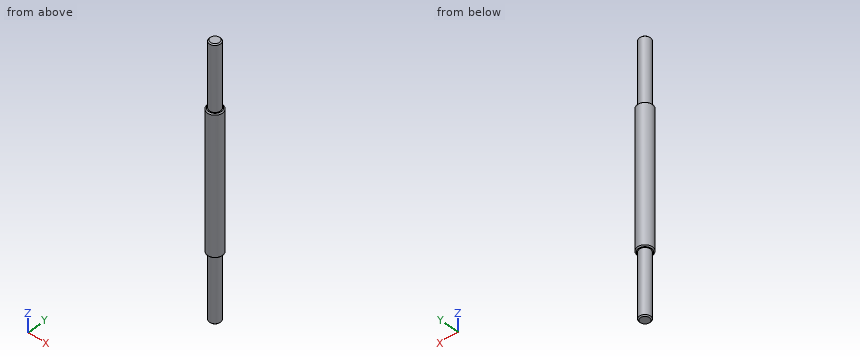
```python
from build123d import *

# Parameters (mm, degrees)
SKETCH1_R           = 7.5
BOSS_EXTRUDE1_DEPTH = 138
SKETCH2_R           = 5.5
BOSS_EXTRUDE2_DEPTH = 20
SKETCH3_R           = 5.5
BOSS_EXTRUDE3_DEPTH = 45
CHAMFER1_SIZE       = 1
BOSS_EXTRUDE4_START = 65
SKETCH4_R           = 5.5
BOSS_EXTRUDE4_DEPTH = 65
CHAMFER2_SIZE       = 1


with BuildPart() as part:
    # Sketch1 → Boss-Extrude1 (new body)
    with BuildSketch(Plane.XY):
        Circle(SKETCH1_R)
    extrude(amount=BOSS_EXTRUDE1_DEPTH)

    # Sketch2 → Boss-Extrude2 (add)
    with BuildSketch(Plane.XY.offset(138)):
        Circle(SKETCH2_R)
    extrude(amount=BOSS_EXTRUDE2_DEPTH)

    # Sketch3 → Boss-Extrude3 (add)
    with BuildSketch(Plane.XY.offset(158)):
        Circle(SKETCH3_R)
    extrude(amount=BOSS_EXTRUDE3_DEPTH)

    # Chamfer1
    chamfer1_edges = [part.edges().sort_by_distance(p)[0] for p in [
        (-7.5, 0, 0),
        (-7.5, 0, 138),
        (-5.5, 0, 203),
    ]]
    chamfer(chamfer1_edges, length=CHAMFER1_SIZE)

    # Sketch4 → Boss-Extrude4 (add)
    with BuildSketch(Plane(origin=(0, 0, 0), x_dir=(-1, 0, 0), z_dir=(0, 0, -1)).offset(BOSS_EXTRUDE4_START)):
        with Locations(Location((0, 0, 0), (0, 0, 180))):
            Circle(SKETCH4_R)
    extrude(amount=-BOSS_EXTRUDE4_DEPTH)

    # Chamfer2
    chamfer2_edges = [part.edges().sort_by_distance(p)[0] for p in [
        (-5.5, 0, -65),
    ]]
    chamfer(chamfer2_edges, length=CHAMFER2_SIZE)


solid = part.part
```
The model under review builds one solid part; all positions refer to its coordinate system, in mm. Coordinates: 2 decimals unless noted, no trailing zeros. Write each loop counter-clockwise with the first axis right and the second up, starting at its lowest first coordinate (ties: lowest second). Pieces come first, ordered by that corner, then holes.
1) We need section A-A on y = 0. State the section outline as (x, z) points.
2) To check wall thickness, follow probe 1 along Z at (x, y) = (-1.25, -5.5); probe 2 along Z at (x, y) = (1.5, 5.25); probe 3 along X at (y, z) = (-0.25, 159). State the ranges of each line that lie inside material, in increasing order.
3) We need section C-C on z = 37. State the section outline as (x, y) points, then the cut area to 3 significant figures.
4) We need section D-D on z = 158. State the section outline as (x, y) points.
5) Clearance check with flat-ended pins moving along their axes: pin 1 Ø8 at (x, z) = (5, 173.5) entering from -Y; pin 2 Ø6 at (x, y) = (-5.5, 4) entering from +Z; pin 3 Ø2 at (x, z) = (0, 166.5) entering from -Y; pin 4 Ø1 at (x, z) = (-3, 93) entering from +Y. State where each tip first meets the part, or that it passes through.
Answer list:
1. outline: (-7.5, 1) - (-6.5, 0) - (-5.5, 0) - (-5.5, -64) - (-4.5, -65) - (4.5, -65) - (5.5, -64) - (5.5, 0) - (6.5, 0) - (7.5, 1) - (7.5, 137) - (6.5, 138) - (5.5, 138) - (5.5, 202) - (4.5, 203) - (-4.5, 203) - (-5.5, 202) - (-5.5, 138) - (-6.5, 138) - (-7.5, 137) - close
2. probe 1: z = 0 to 138
2. probe 2: z = -64.04 to 202.04
2. probe 3: x = -5.49 to 5.49
3. outline: circle Ø15 at (0, 0)
3. area: 177 mm2
4. outline: circle Ø11 at (0, 0)
5. pin 1: stops at y = -5.41
5. pin 2: stops at z = 203
5. pin 3: stops at y = -5.5
5. pin 4: stops at y = 7.07
